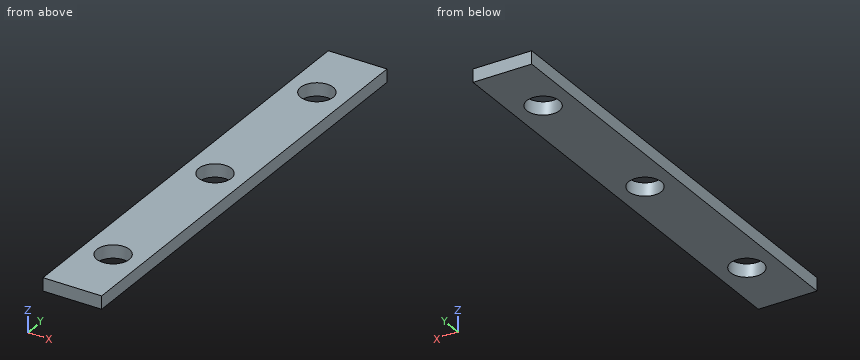
from build123d import *

# Parameters (mm, degrees)
SKETCH_1_W          = 18
SKETCH_1_H          = 140
SKETCH_1_R          = 5
BOSS_EXTRUDE1_DEPTH = 4


with BuildPart() as part:
    # Sketch 1 → Boss-Extrude1 (new body)
    with BuildSketch(Plane.XY):
        Rectangle(SKETCH_1_W, SKETCH_1_H)
        with Locations((0, 50)):
            Circle(SKETCH_1_R, mode=Mode.SUBTRACT)
        Circle(SKETCH_1_R, mode=Mode.SUBTRACT)
        with Locations((0, -50)):
            Circle(SKETCH_1_R, mode=Mode.SUBTRACT)
    extrude(amount=BOSS_EXTRUDE1_DEPTH)


solid = part.part
Geometry: final body of the model. Coordinates: model frame, mm. Give positions to 0.01 mm unless a question says otherwise; leave off trailing zeros. Loops run counter-clockwise (first coordinate to the right, second up) from the corner with the lowest first, then second, coordinate; pieces in that order, holes last. Notation, with made-up numbers: (62, 52) - (68, 52) arc R17 cw to (68, 61) - close; hole circle Ø8 at (-22.5, -35). An arc over 180 degrees is marked (long way). Answer as CSV lines item,"result". Start each with the question number.
1. Ray query, L1, parallel to Y at x = 0, z = 2.65; L2, parallel to Y at x = 4, z = 1.3; L3, parallel to X at y = -49.5, z = 1.9. Return the intervals inside material, ascending.
2. Section A-A, the plane x = 0. Return loops of the section in (y, z), plus the area to 3 significant figures.
3. Section C-C, the plane z = 2.4. Return loops of the section in (x, y), plus the area to 3 significant figures.
4. Section B-B, the plane y = 0. Return loops of the section in (x, z), plus the area to 3 significant figures.
5. Pin query (flat end, axial travel): P1, Ø6, axis at x = 2, y = 24.5, coming from the -Z side. Return the tip coordinate at first contact, or that it passes through.
Answers:
1,L1,"y = -70 to -55, -45 to -5, 5 to 45, 55 to 70"
1,L2,"y = -70 to -53, -47 to -3, 3 to 47, 53 to 70"
1,L3,"x = -9 to -4.97, 4.97 to 9"
2,outline,"(-70, 0) - (-55, 0) - (-55, 4) - (-70, 4) - close; (-45, 0) - (-5, 0) - (-5, 4) - (-45, 4) - close; (5, 0) - (45, 0) - (45, 4) - (5, 4) - close; (55, 0) - (70, 0) - (70, 4) - (55, 4) - close"
2,area,"440 mm2"
3,outline,"(-9, -70) - (9, -70) - (9, 70) - (-9, 70) - close; hole circle Ø10 at (0, -50); hole circle Ø10 at (0, 0); hole circle Ø10 at (0, 50)"
3,area,"2,280 mm2"
4,outline,"(-9, 0) - (-5, 0) - (-5, 4) - (-9, 4) - close; (5, 0) - (9, 0) - (9, 4) - (5, 4) - close"
4,area,"32.0 mm2"
5,P1,"stops at z = 0"
